Read the model definition and answer for the solid it produces. Units are mm, in the model's axes. Give positions to 0.01 mm unless a question says otherwise; leave off trailing zeros. Order: outer loops, then holes, each group sorted by start corner. A loop starts at its lowest first (then second) coordinate and runs counter-clockwise, first axis right, second up. Notation, with made-up numbers: (-23.5, -24) -> (19.5, -24) arc R18 ccw to (19.5, -7) -> close; hole circle Ø8 at (-8.5, -39). An arc over 180 degrees is marked (long way). Use one line per item in the form item = value.
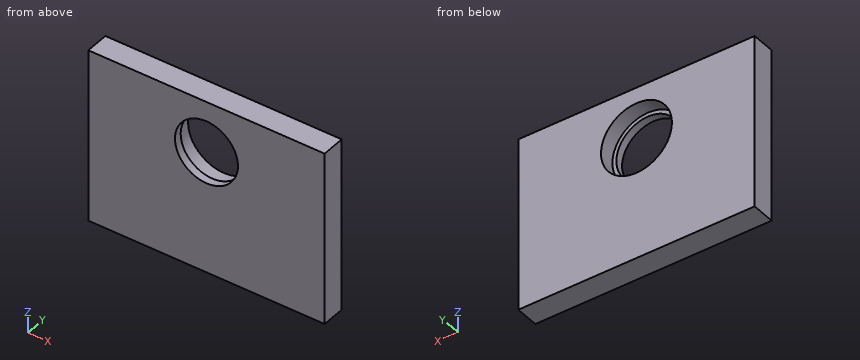
```python
from build123d import *

# Parameters (mm, degrees)
SKETCH_1_W          = 300
SKETCH_1_H          = 220
EXTRUDE_1_DEPTH     = 30
SKETCH_2_R          = 45
CUT_EXTRUDE_1_DEPTH = 20
SKETCH_3_R          = 40
CUT_EXTRUDE_2_DEPTH = 189.414436814


with BuildPart() as part:
    # 草图1 → 凸台-拉伸1 (new body)
    with BuildSketch(Plane(origin=(0, 0, 0), x_dir=(1, 0, 0), z_dir=(0, 1, 0))):
        Rectangle(SKETCH_1_W, SKETCH_1_H)
    extrude(amount=EXTRUDE_1_DEPTH)

    # 草图2 → 切除-拉伸1 (cut)
    with BuildSketch(Plane(origin=(0, 30, 0), x_dir=(1, 0, 0), z_dir=(0, 1, 0))):
        with Locations(Location((0, -45, 0), (0, 0, 270))):
            Circle(SKETCH_2_R)
    extrude(amount=-CUT_EXTRUDE_1_DEPTH, mode=Mode.SUBTRACT)

    # 草图3 → 切除-拉伸2 (cut, through all)
    with BuildSketch(Plane(origin=(0, 30, 0), x_dir=(1, 0, 0), z_dir=(0, 1, 0))):
        with Locations(Location((0, -45, 0), (0, 0, 270))):
            Circle(SKETCH_3_R)
    extrude(amount=-CUT_EXTRUDE_2_DEPTH, mode=Mode.SUBTRACT)


solid = part.part
```
Item 1: The part is cut by section B-B on x = 0. Give the vertices of the cut face in (y, z), and give its area (3 significant figures).
Checks:
outline = (0, -110) -> (30, -110) -> (30, 0) -> (10, 0) -> (10, 5) -> (0, 5) -> close; (0, 85) -> (10, 85) -> (10, 90) -> (30, 90) -> (30, 110) -> (0, 110) -> close
area = 4,000 mm²
Item 2: The part is cut by section A-A on z = 45. Give the vertices of the cut face in (x, y), and give its area (3 significant figures).
Checks:
outline = (-150, 0) -> (-40, 0) -> (-40, 10) -> (-45, 10) -> (-45, 30) -> (-150, 30) -> close; (40, 0) -> (150, 0) -> (150, 30) -> (45, 30) -> (45, 10) -> (40, 10) -> close
area = 6,400 mm²
Item 3: Straight lines are drawn through the part: L1, parallel to X at y = 24.75, z = 45; L2, parallel to Z at x = -27, y = 23.5; L3, parallel to Z at x = 17.5, y = 11.75. For each, find the intervals that lie inside material, in ascending order. Write a range as from..to.
Checks:
L1 = -150..-45, 45..150
L2 = -110..9, 81..110
L3 = -110..3.54, 86.46..110
Item 4: The part is cut by section C-C on y = 15. Give the vertices of the cut face in (x, z).
Checks:
outline = (-150, -110) -> (150, -110) -> (150, 110) -> (-150, 110) -> close; hole circle Ø90 at (0, 45)
